Input: dimensioned drawing with shaded views. Units: mm. Origin: part minimum x, y, z. A direction names the side the tool comes from. Give positions to 0.01 mm unless a question says otherwise; leave off trailing zeros. Loops run counter-clockwise (first coordinate to the right, second up) from the corner with the lowest first, then second, coordinate; pieces in that order, holes last.
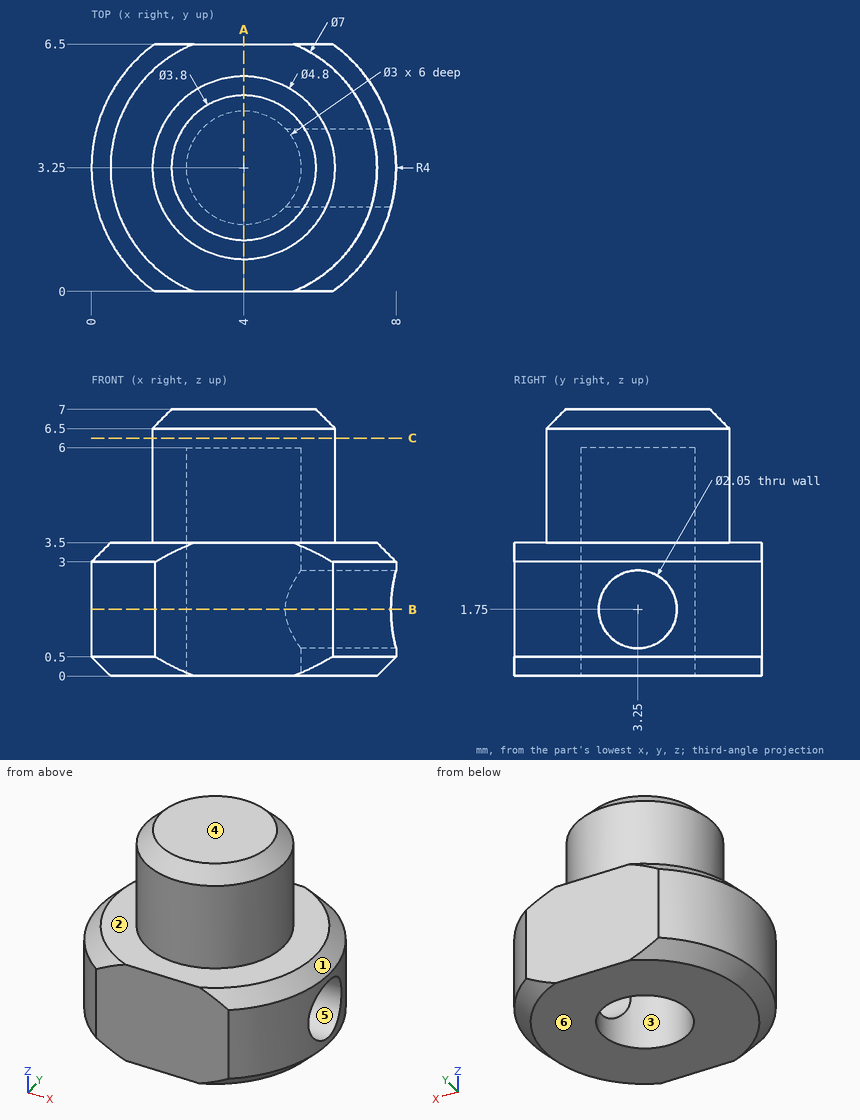
(1) Reachability of the marked faces 1, 2 and 3 from +Z, -Z, +X, -X, +Y, -Y: full face, straight path, thin tool, end or side. Return the list, or none.
A:
face 1: +Z, +X
face 2: +Z
face 3: -Z
(2) Section C-C, the plane z = 6.25. Return the cut outline in (x, y).
A:
outline: circle Ø4.8 at (4, 3.25)
(3) First-contact query: pin 1 (1 mm diameter, centred on y = 3.5, z = 5.5, fed in from +X); pin 2 (1 mm diameter, centred on y = 4.5, z = 5, fed in from +X). Flat tips, straight axial feed; report the tip coordinate or a pass-through.
A:
pin 1: stops at x = 6.4
pin 2: stops at x = 6.28
(4) Ray query, line 1 along Y through (x, z) = (4, 4.75); line 2 along Y through (x, z) = (7.2, 1.75) (3 decimals); line 3 along Z through (x, y) = (4, 0.75). Return the intervals inside material, ascending.
A:
line 1: y = 0.85 to 1.75, 4.75 to 5.65
line 2: y = 0.85 to 2.225, 4.275 to 5.65
line 3: z = 0 to 3.5
(5) Mould query, pull axis Z, two halves, no side actions, for the marked faces 4, 5 and 6. Classes: pulls with the +Z half, pulls with the -Z half, needs draft (parallel to the pull), parting line crosses it, or undercut.
A:
face 4: pulls with the +Z half
face 5: undercut
face 6: pulls with the -Z half
(6) Section B-B, the plane z = 1.75. Return the cut outline in (x, y) (3 decimals).
A:
outline: (1.668, 0) - (6.332, 0) arc R4 ccw to (7.866, 2.225) - (5.095, 2.225) arc R1.5 cw (long way) to (5.095, 4.275) - (7.866, 4.275) arc R4 ccw to (6.332, 6.5) - (1.668, 6.5) arc R4 ccw to start
(7) Section A-A, the plane x = 4. Return the cut outline in (y, z).
A:
outline: (0, 0) - (1.75, 0) - (1.75, 6) - (4.75, 6) - (4.75, 0) - (6.5, 0) - (6.5, 3.5) - (5.65, 3.5) - (5.65, 6.5) - (5.15, 7) - (1.35, 7) - (0.85, 6.5) - (0.85, 3.5) - (0, 3.5) - close
